Build history of the part. All positions in model axes, mm. Coordinates: 2 decimals unless noted, no trailing zeros. Loops run counter-clockwise (first coordinate to the right, second up) from the corner with the lowest first, then second, coordinate; pieces in that order, holes last.
(1) Slice it at B-B (x = 10). Give the cut face in (y, z).
(2) Wall check: L1, parallel to Z at x = 5, y = 208; L2, parallel to Z at x = -20.5, y = 960. Give the ranges that are in metal, low to high.
(3) Slice it at C-C (y = 639). Give the cut face in (x, z), and give its area (3 significant figures).
(4) Slice it at A-A (z = -10). Give the cut face in (x, y), and give its area (3 significant figures).
from build123d import *

# Parameters (mm, degrees)
EXTRUDE_1_DEPTH = 1550


with BuildPart() as part:
    # 草图1 → 凸台-拉伸1 (new body)
    with BuildSketch(Plane(origin=(0, 0, 0), x_dir=(1, 0, 0), z_dir=(0, 1, 0))):
        with BuildLine():
            Line((-19, -25), (19, -25))
            ThreePointArc((19, -25), (23.242640687, -23.242640687), (25, -19))
            Line((25, -19), (25, 19))
            ThreePointArc((25, 19), (23.242640687, 23.242640687), (19, 25))
            Line((19, 25), (-19, 25))
            ThreePointArc((-19, 25), (-23.242640687, 23.242640687), (-25, 19))
            Line((-25, 19), (-25, -19))
            ThreePointArc((-25, -19), (-23.242640687, -23.242640687), (-19, -25))
        make_face()
        with BuildLine():
            Line((-19, -20), (19, -20))
            ThreePointArc((19, -20), (19.707106781, -19.707106781), (20, -19))
            Line((20, -19), (20, 19))
            ThreePointArc((20, 19), (19.707106781, 19.707106781), (19, 20))
            Line((19, 20), (-19, 20))
            ThreePointArc((-19, 20), (-19.707106781, 19.707106781), (-20, 19))
            Line((-20, 19), (-20, -19))
            ThreePointArc((-20, -19), (-19.707106781, -19.707106781), (-19, -20))
        make_face(mode=Mode.SUBTRACT)
    extrude(amount=EXTRUDE_1_DEPTH)


solid = part.part
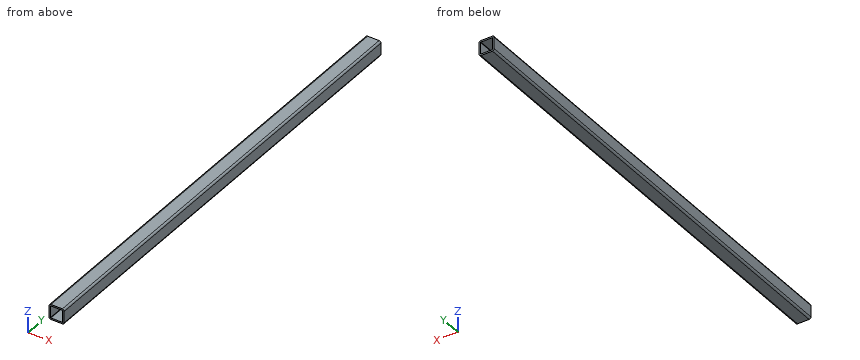
Response values:
1. outline: (0, -25) - (1550, -25) - (1550, -20) - (0, -20) - close; (0, 20) - (1550, 20) - (1550, 25) - (0, 25) - close
2. L1: z = -25 to -20, 20 to 25
2. L2: z = -24.81 to 24.81
3. outline: (-25, -19) arc R6 ccw to (-19, -25) - (19, -25) arc R6 ccw to (25, -19) - (25, 19) arc R6 ccw to (19, 25) - (-19, 25) arc R6 ccw to (-25, 19) - close; hole (-20, -19) arc R1 ccw to (-19, -20) - (19, -20) arc R1 ccw to (20, -19) - (20, 19) arc R1 ccw to (19, 20) - (-19, 20) arc R1 ccw to (-20, 19) - close
3. area: 870 mm2
4. outline: (-25, 0) - (-20, 0) - (-20, 1550) - (-25, 1550) - close; (20, 0) - (25, 0) - (25, 1550) - (20, 1550) - close
4. area: 15,500 mm2
